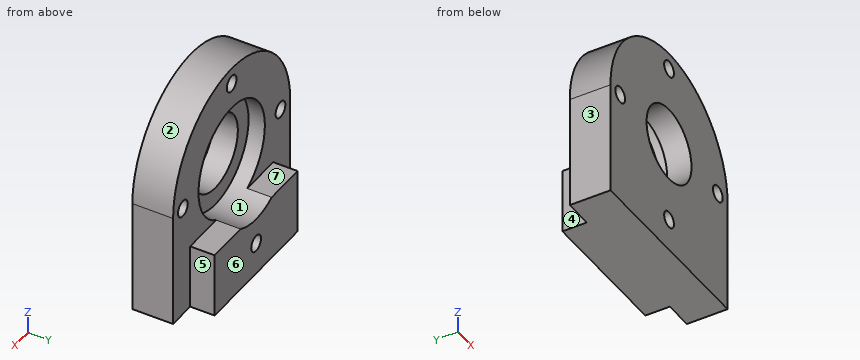
```python
from build123d import *

# Parameters (mm, degrees)
BASE_PLATE_DEPTH          = 25
UPRIGHT_BLOCK_SKETCH_W    = 85
UPRIGHT_BLOCK_SKETCH_H    = 15
UPRIGHT_BLOCK_DEPTH       = 40
MOUNTING_HOLES_SKETCH_R   = 5
MOUNTING_HOLES_CUT_DEPTH  = 40
COUNTERBORE_68_DEPTH      = 40
COUNTERBORE_68_DEPTH_BACK = 10
COUNTERBORE_68_SKETCH_R   = 34
BORE_46_SKETCH_R          = 23
BORE_46_DEPTH             = 15


with BuildPart() as part:
    # Base Plate Sketch → Base Plate (new body)
    with BuildSketch(Plane(origin=(0, 0, 0), x_dir=(1, 0, 0), z_dir=(0, 1, 0))):
        with BuildLine():
            Line((-60, 35), (60, 35))
            Line((60, 35), (60, -35))
            ThreePointArc((60, -35), (0, -95), (-60, -35))
            Line((-60, -35), (-60, 35))
        make_face()
    extrude(amount=BASE_PLATE_DEPTH)

    # Upright Block Sketch → Upright Block (add)
    with BuildSketch(Plane(origin=(0, 0, -35), x_dir=(-1, 0, 0), z_dir=(0, 0, -1))):
        with Locations((0, 32.5)):
            Rectangle(UPRIGHT_BLOCK_SKETCH_W, UPRIGHT_BLOCK_SKETCH_H)
    extrude(amount=-UPRIGHT_BLOCK_DEPTH)

    # Mounting Holes Sketch → Mounting Holes Cut (cut)
    with BuildSketch(Plane(origin=(0, 40, 0), x_dir=(1, 0, 0), z_dir=(0, 1, 0))):
        with Locations(Location((0, 15, 0), (0, 0, 270))):
            Circle(MOUNTING_HOLES_SKETCH_R)
        with Locations(Location((-50, -35, 0), (0, 0, 270))):
            Circle(MOUNTING_HOLES_SKETCH_R)
        with Locations(Location((50, -35, 0), (0, 0, 270))):
            Circle(MOUNTING_HOLES_SKETCH_R)
        with Locations(Location((0, -85, 0), (0, 0, 270))):
            Circle(MOUNTING_HOLES_SKETCH_R)
    extrude(amount=-MOUNTING_HOLES_CUT_DEPTH, mode=Mode.SUBTRACT)

    # Counterbore Ø68 Sketch → Counterbore Ø68 (cut, two sides: drawn at the far end of the back side and taken through both)
    with BuildSketch(Plane(origin=(0, 25, 0), x_dir=(1, 0, 0), z_dir=(0, 1, 0)).offset(-COUNTERBORE_68_DEPTH_BACK)):
        with Locations(Location((0, -35, 0), (0, 0, 61.927513064))):
            Circle(COUNTERBORE_68_SKETCH_R)
    extrude(amount=COUNTERBORE_68_DEPTH + COUNTERBORE_68_DEPTH_BACK, mode=Mode.SUBTRACT)

    # Bore Ø46 Sketch → Bore Ø46 (cut)
    with BuildSketch(Plane(origin=(0, 15, 0), x_dir=(1, 0, 0), z_dir=(0, 1, 0))):
        with Locations(Location((0, -35, 0), (0, 0, 270))):
            Circle(BORE_46_SKETCH_R)
    extrude(amount=-BORE_46_DEPTH, mode=Mode.SUBTRACT)


solid = part.part
```
Could you check a few things on this model? Use its own coordinates, in mm. Face numbers are marked on the shaded views. A direction names the side the tool comes from. Round coordinates to 2 decimals unless told otherwise and drop trailing zeros. Loops run counter-clockwise (first coordinate to the right, second up) from the corner with the lowest first, then second, coordinate; pieces in that order, holes last. Notation, with made-up numbers: M -17,22.25 L 20,22.25 A19 cw 20,57.25 Z; hole C 62,2.25 d6. An arc over 180 degrees is marked long. Answer as CSV lines item,"result".
1) Which directions (+Z, -Z, +X, -X, +Y, -Y) give clear straight access to the entire face, cutting with the end or side of a thin tool? Please do the marked faces 4, 5, 6 and 7.
From the geometry:
face 4,"+Z, -Z, -X, +Y"
face 5,"+Z, -Z, +X, +Y"
face 6,"+Z, -Z, +X, -X, +Y"
face 7,"+Z, +X, -X, +Y"
2) Imagine slicing it at C-C on x = 17.5. List the corners of the cut face in (y, z) for me, and give its area (3 significant figures).
From the geometry:
outline,"M 0,-35 L 40,-35 L 40,5 L 25,5 L 25,5.85 L 15,5.85 L 15,20.08 L 0,20.08 Z; M 0,49.92 L 15,49.92 L 15,64.15 L 25,64.15 L 25,92.39 L 0,92.39 Z"
area,"2,750 mm^2"
3) Imagine slicing it at A-A on z = -18. List the corners of the cut face in (x, y) for me, and give its area (4 significant figures).
From the geometry:
outline,"M -60,0 L -4,0 L -4,40 L -42.5,40 L -42.5,25 L -60,25 Z; M 4,0 L 60,0 L 60,25 L 42.5,25 L 42.5,40 L 4,40 Z"
area,"3,955 mm^2"
4) Imagine slicing it at D-D on y = 33. List the corners of the cut face in (x, z) for me.
From the geometry:
outline,"M -42.5,-35 L 42.5,-35 L 42.5,5 L 16,5 A34 cw -16,5 L -42.5,5 Z; hole C 0,-15 d10"
5) Imagine slicing it at B-B on y = 6. List the corners of the cut face in (x, z) for me.
From the geometry:
outline,"M -60,-35 L 60,-35 L 60,35 A60 ccw -60,35 Z; hole C -50,35 d10; hole C 0,35 d46; hole C 0,-15 d10; hole C 0,85 d10; hole C 50,35 d10"
6) If I drill on probe 1 along X at (y, z) = (27, -15); probe 2 along X at (y, z) = (18, 34); probe 3 along Z at (x, y) = (-4.5, 5), over which ranges is the centre line in solid material (lowest first)?
From the geometry:
probe 1,"-42.5 to -5, 5 to 42.5"
probe 2,"-60 to -54.9, -45.1 to -33.99, 33.99 to 45.1, 54.9 to 60"
probe 3,"-35 to -17.18, -12.82 to 12.44, 57.56 to 82.82, 87.18 to 94.83"
7) We'd pull the mould along Z, two halves only. Please class the marked faces 1, 2 and 3: released by +Z, released by -Z, zero draft, split by the parting line, or undercut.
From the geometry:
face 1,"undercut"
face 2,"released by +Z"
face 3,"zero draft"
8) For pin 1 Ø8 at (y, z) = (7.5, 65.5) entering from -X; pin 2 Ø7.5 at (y, z) = (33, -20.5) entering from -X; pin 3 Ø7.5 at (x, y) = (23.5, 29) entering from +Z, each with a flat end and sliding along its axis, tell me the tip position at first contact or that it passes through.
From the geometry:
pin 1,"x = -53.83"
pin 2,"x = -42.5"
pin 3,"z = 5"
